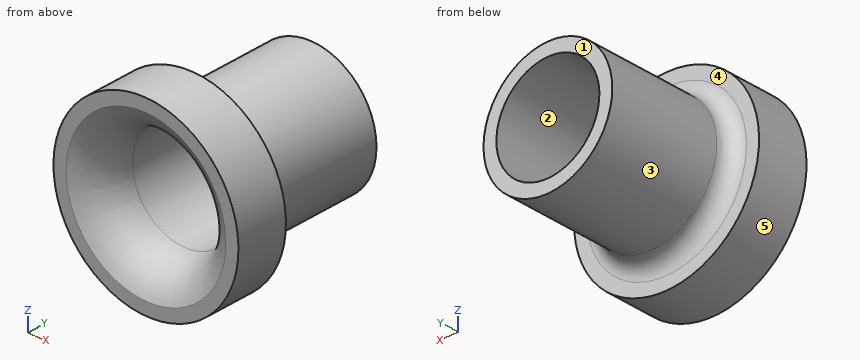
from build123d import *


with BuildPart() as part:
    # Sketch1 → Revolve2 (revolve)
    with BuildSketch(Plane.XY, mode=Mode.PRIVATE) as revolve2_sk:
        with BuildLine():
            Line((-10, 28.836781592), (-12.5, 28.836781592))
            Line((-12.5, 28.836781592), (-12.5, 6.836781592))
            ThreePointArc((-12.5, 6.836781592), (-13.378679656, 4.715461249), (-15.5, 3.836781592))
            Line((-15.5, 3.836781592), (-17.956309532, 3.836781592))
            Line((-17.956309532, 3.836781592), (-17.956309532, -6.163218408))
            Line((-17.956309532, -6.163218408), (-15.5, -6.163218408))
            ThreePointArc((-15.5, -6.163218408), (-11.507640786, -3.017340367), (-10, 1.836781592))
            Line((-10, 1.836781592), (-10, 28.836781592))
        make_face()
    revolve(revolve2_sk.sketch.rotate(Axis((0, 10.886363636, 0), (0, -1, 0)), 270), axis=Axis((0, 10.886363636, 0), (0, -1, 0)))


solid = part.part
Work out the finished part from the listing and answer in its coordinate system (mm). Face numbers are marked on the shaded views. A direction names the side the tool comes from. Round coordinates to 2 decimals unless told otherwise and drop trailing zeros. Order: outer loops, then holes, each group sorted by start corner. A loop starts at its lowest first (then second) coordinate and runs counter-clockwise, first axis right, second up. Notation, with made-up numbers: M 33,49.25 L 79,49.25 A16 cw 79,61.25 Z; hole C 61.5,72 d8. An arc over 180 degrees is marked long. Put each result on its own line as item: value. Start each with the question number.
Q1. Section A-A, the plane x = 0 is taken. Write down the section's boundary in (y, z).
Q2. A tool of negligible diameter and unlimited length cuts with its end or side. For the marked faces 4 and 5, from which of +Z, -Z, +X, -X, +Y, -Y can it reach the whole face along a straight path? Write none if from no direction.
Q3. For a pull along X with two mould halves and no side action, classify the marked faces 1, 2 and 3 as pulls with the +X half, pulls with the -X half, needs draft (parallel to the pull), parting line crosses it, or undercut.
Q4. Flat-ended cylindrical pins translate along their axes: pin 1 (4 mm diameter, centred on x = 1, y = 22.5, fed in from -Z); pin 2 (1.5 mm diameter, centred on x = -11.5, y = 14, fed in from +Z); pin 3 (12 mm diameter, centred on y = 2, z = 13.5, fed in from +X) (3 decimals). Find the tip coordinate at first contact, or state that the pin passes through.
Q5. Section B-B, the plane z = 0 is taken. Write down the section's boundary in (x, y), and give its area (3 significant figures).
Q6. Section C-C, the plane y = 2.5 is taken. Write down the section's boundary in (x, z).
Q7. Straight lines are drawn through the part: L1, parallel to X at y = 17.25, z = 0; L2, parallel to Y at x = 16.5, z = 1.5; L3, parallel to Z at x = -6.5, y = 7. For each, find the intervals that lie inside material, in ascending order. Write a range as [from, to].
Findings below:
1. outline: M -6.16,-17.96 L 3.84,-17.96 L 3.84,-15.5 A3 cw 6.84,-12.5 L 28.84,-12.5 L 28.84,-10 L 1.84,-10 A8.57 ccw -6.16,-15.5 Z; M -6.16,15.5 A8.57 ccw 1.84,10 L 28.84,10 L 28.84,12.5 L 6.84,12.5 A3 cw 3.84,15.5 L 3.84,17.96 L -6.16,17.96 Z
2. face 4: +Y
2. face 5: +Y, -Y
3. face 1: needs draft
3. face 2: undercut
3. face 3: parting line crosses it
4. pin 1: stops at z = -12.5
4. pin 2: stops at z = 6.38
4. pin 3: stops at x = 16.315
5. outline: M -17.96,-6.16 L -15.5,-6.16 A8.57 ccw -10,1.84 L -10,28.84 L -12.5,28.84 L -12.5,6.84 A3 cw -15.5,3.84 L -17.96,3.84 Z; M 10,1.84 A8.57 ccw 15.5,-6.16 L 17.96,-6.16 L 17.96,3.84 L 15.5,3.84 A3 cw 12.5,6.84 L 12.5,28.84 L 10,28.84 Z
5. area: 264 mm^2
6. outline: C 0,0 d35.91; hole C 0,0 d20
7. L1: x = [-12.5, -10], [10, 12.5]
7. L2: y = [-6.16, 3.84]
7. L3: z = [-10.68, -7.6], [7.6, 10.68]
